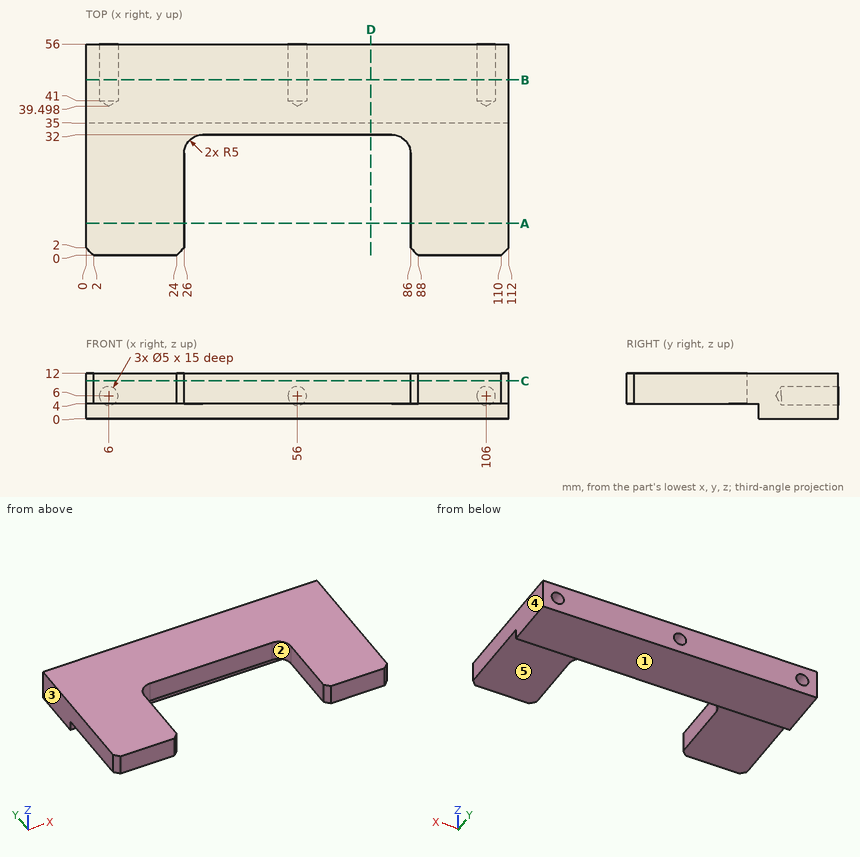
Input: dimensioned drawing with shaded views. Units: mm. Origin: part minimum x, y, z. A direction names the side the tool comes from. Give positions to 0.01 mm unless a question says otherwise; leave off trailing zeros. Order: outer loops, then holes, each group sorted by start corner. A loop starts at its lowest first (then second) coordinate and runs counter-clockwise, first axis right, second up. Notation, with made-up numbers: (37, 86.25) -> (62, 86.25) arc R13 cw to (62, 99.25) -> close; hole circle Ø11 at (-29.75, -9). An arc over 180 degrees is marked (long way). Use a Markdown table: item, result.
1) Section query A-A, the plane y = 8.5. Return the cut outline in (x, z), then the cut area to 3 significant figures.
Answer list:
| item | result |
|---|---|
| outline | (0, 4) -> (26, 4) -> (26, 12) -> (0, 12) -> close; (86, 4) -> (112, 4) -> (112, 12) -> (86, 12) -> close |
| area | 416 mm² |
2) Mould query, pull axis X, two halves, no side actions, for the marked faces 1, 2 and 3. Classes: +X half, -X half, draft (parallel to the pull), parting line (faces both ways), or undercut.
Answer list:
| item | result |
|---|---|
| face 1 | draft |
| face 2 | undercut |
| face 3 | -X half |
3) Ray query, line 1 along X through (y, z) = (4, 4.5); line 2 along Z through (x, y) = (106, 46); line 3 along X through (y, z) = (42, 6.75) (1 decimal). Return the intervals inside material, ascending. Write a range as [from, to].
Answer list:
| item | result |
|---|---|
| line 1 | [0, 26], [86, 112] |
| line 2 | [0, 3.5], [8.5, 12] |
| line 3 | [0, 3.6], [8.4, 53.6], [58.4, 103.6], [108.4, 112] |
4) Section query B-B, the plane y = 46.5. Return the cut outline in (x, z), then the cut area to 3 significant figures.
Answer list:
| item | result |
|---|---|
| outline | (0, 0) -> (112, 0) -> (112, 12) -> (0, 12) -> close; hole circle Ø5 at (6, 6); hole circle Ø5 at (56, 6); hole circle Ø5 at (106, 6) |
| area | 1,290 mm² |
5) Contact query for flat-ended pins moving along their axis: P1, Ø4.5, axis at x = 106, z = 6, coming from the +Y side; P2, Ø1, axis at x = 51.5, z = 5, coming from the -Y side; P3, Ø1, axis at x = 45.5, z = 1, coming from the -Y side; P4, Ø6, axis at x = 56, z = 6, coming from the +Y side. Output: stop coordinate, or through.
Answer list:
| item | result |
|---|---|
| P1 | y = 40.85 |
| P2 | y = 32 |
| P3 | y = 35 |
| P4 | y = 56 |
6) Section query D-D, the plane x = 75.5. Return the cut outline in (y, z).
Answer list:
| item | result |
|---|---|
| outline | (32, 4) -> (35, 4) -> (35, 0) -> (56, 0) -> (56, 12) -> (32, 12) -> close |
7) Reachability of the marked faces 4 and 5 from +Z, -Z, +X, -X, +Y, -Y: full face, straight path, thin tool, end or side. Return the list, or none.
Answer list:
| item | result |
|---|---|
| face 4 | +Z, -Z, +X, +Y, -Y |
| face 5 | -Z, +X, -X, -Y |
8) Section query C-C, the plane z = 10. Return the cut outline in (x, y).
Answer list:
| item | result |
|---|---|
| outline | (0, 2) -> (2, 0) -> (24, 0) -> (26, 2) -> (26, 27) arc R5 cw to (31, 32) -> (81, 32) arc R5 cw to (86, 27) -> (86, 2) -> (88, 0) -> (110, 0) -> (112, 2) -> (112, 56) -> (0, 56) -> close |
